Part print with two shaded views. Sizes in mm from the minimum x, y, z corner. Round coordinates to 2 decimals unless told otherwise and drop trailing zeros. Write each loop counter-clockwise with the first axis right and the second up, starting at its lowest first coordinate (ties: lowest second). Pieces come first, ordered by that corner, then holes.
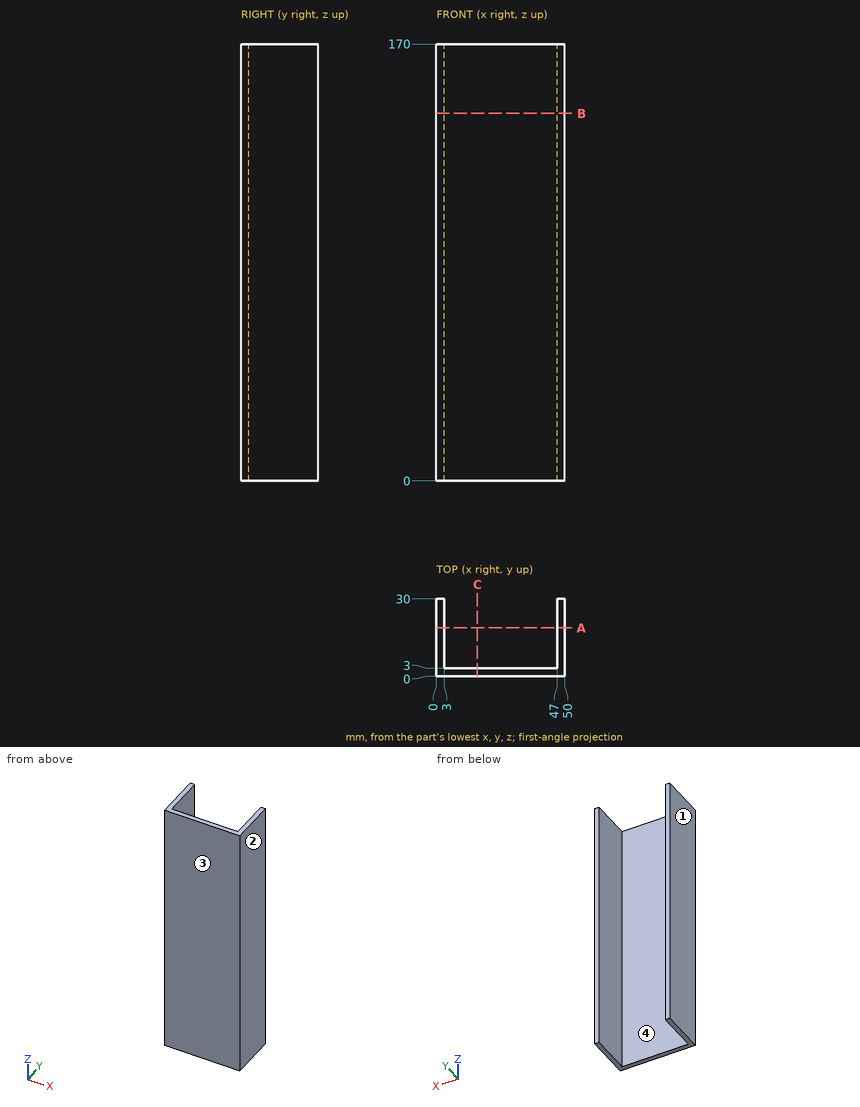
Q1. Wall check: L1, parallel to X at y = 3.75, z = 66; L2, parallel to Y at x = 3.5, z = 62. Give the ranges that are in metal, low to high.
Values follow:
L1: x = 0 to 3, 47 to 50
L2: y = 0 to 3
Q2. Cut at A-A on y = 18.75. Write the cut outline in (x, z), plus the area to 3 significant figures.
Values follow:
outline: (0, 0) - (3, 0) - (3, 170) - (0, 170) - close; (47, 0) - (50, 0) - (50, 170) - (47, 170) - close
area: 1,020 mm2
Q3. Cut at C-C on x = 16. Write the cut outline in (y, z).
Values follow:
outline: (0, 0) - (3, 0) - (3, 170) - (0, 170) - close
Q4. Cut at B-B on z = 143. Write the cut outline in (x, y).
Values follow:
outline: (0, 0) - (50, 0) - (50, 30) - (47, 30) - (47, 3) - (3, 3) - (3, 30) - (0, 30) - close
Q5. Mould opens along X. For the marked faces 1, 2, 3 and 4 say: +X half, -X half, draft (parallel to the pull), parting line (faces both ways), or undercut.
Values follow:
face 1: -X half
face 2: +X half
face 3: draft
face 4: undercut
